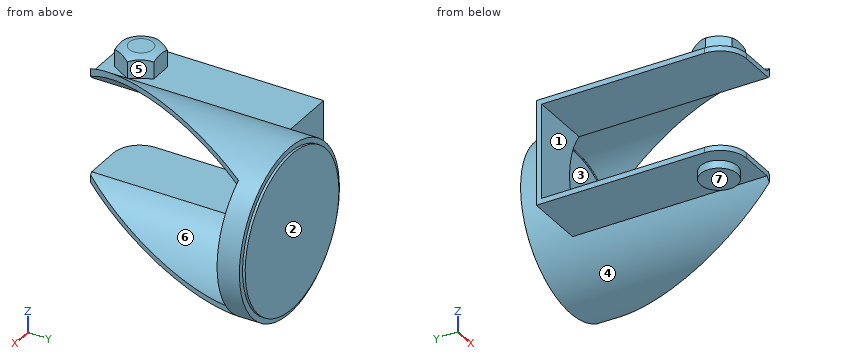
from build123d import *

# Parameters (mm, degrees)
SKETCH2_W               = 36
SKETCH2_H               = 106
CUT_EXTRUDE1_DEPTH      = 95
BOSS_EXTRUDE1_DEPTH     = 47.5
SKETCH4_R               = 29.766666667
CUT_EXTRUDE2_DEPTH      = 144
CUT_EXTRUDE3_DEPTH      = 95
CUT_EXTRUDE3_DEPTH_BACK = 95
SKETCH6_R               = 7
BOSS_EXTRUDE2_DEPTH     = 3
SKETCH8_R               = 9
CUT_EXTRUDE4_DEPTH      = 10


with BuildPart() as part:
    # Sketch1 → Revolve1 (revolve)
    with BuildSketch(Plane(origin=(0, 0, 0), x_dir=(0, 0, -1), z_dir=(1, 0, 0))):
        Polygon((0, -17.975), (-29.666666667, -17.975), (-29.666666667, -109.475), (-31.666666667, -109.475), (-31.666666667, -16.475), (-29.666666667, -16.475), (-29.666666667, -15.475), (0, -15.475), align=None)
    revolve(axis=Axis((0, -15.475, 0), (0, -1, 0)))

    # Sketch2 → Cut-Extrude1 (cut)
    with BuildSketch(Plane(origin=(0, 0, 0), x_dir=(0, 0, -1), z_dir=(1, 0, 0))):
        with Locations((0, -87)):
            Rectangle(SKETCH2_W, SKETCH2_H)
    extrude(amount=-CUT_EXTRUDE1_DEPTH, mode=Mode.SUBTRACT)

    # Sketch3 → Boss-Extrude1 (add)
    with BuildSketch(Plane(origin=(0, 0, 0), x_dir=(0, 0, -1), z_dir=(1, 0, 0))):
        Polygon((-20, -32), (-20, -106), (-18, -106), (-18, -34), (18, -34), (18, -106), (20, -106), (20, -32), align=None)
    extrude(amount=-BOSS_EXTRUDE1_DEPTH)

    # Sketch4 → Cut-Extrude2 (cut)
    with BuildSketch(Plane(origin=(0, -18.475, 0), x_dir=(1, 0, 0), z_dir=(0, 1, 0))):
        with Locations(Location((0, 0, 0), (0, 0, 270))):
            Circle(SKETCH4_R)
    extrude(amount=-CUT_EXTRUDE2_DEPTH, mode=Mode.SUBTRACT)

    # Sketch5 → Cut-Extrude3 (cut, two sides: drawn at the far end of the back side and taken through both)
    with BuildSketch(Plane.XY.offset(-CUT_EXTRUDE3_DEPTH_BACK)):
        with BuildLine():
            Line((-81.666666667, -159.475), (31.666666667, -159.475))
            Line((31.666666667, -159.475), (31.666666667, -24.975))
            Line((31.666666667, -24.975), (18.095238095, -24.975))
            Line((18.095238095, -24.975), (-23.03030303, -106))
            Line((-23.03030303, -106), (-37.5, -106))
            ThreePointArc((-37.5, -106), (-44.571067812, -103.071067812), (-47.5, -96))
            Line((-47.5, -96), (-47.5, -61.653061224))
            Line((-47.5, -61.653061224), (-81.666666667, -106))
            Line((-81.666666667, -106), (-81.666666667, -159.475))
        make_face()
    extrude(amount=CUT_EXTRUDE3_DEPTH + CUT_EXTRUDE3_DEPTH_BACK, mode=Mode.SUBTRACT)

    # Sketch6 → Boss-Extrude2 (add)
    with BuildSketch(Plane.XY.offset(-20)):
        with Locations((-35, -94)):
            Circle(SKETCH6_R)
    extrude(amount=-BOSS_EXTRUDE2_DEPTH)

    # Sketch7 → Revolve2 (revolve)
    with BuildSketch(Plane(origin=(-35, 0, 0), x_dir=(0, 0, -1), z_dir=(1, 0, 0)), mode=Mode.PRIVATE) as revolve2_sk:
        with BuildLine():
            Line((-28, -94), (-28, -89.5))
            ThreePointArc((-28, -89.5), (-27.442646012, -87.053268439), (-26, -85))
            Line((-26, -85), (-20, -85))
            Line((-20, -85), (-20, -94))
            Line((-20, -94), (-28, -94))
        make_face()
    revolve(revolve2_sk.sketch.rotate(Axis((-35, -94, 20), (0, 0, 1)), 90), axis=Axis((-35, -94, 20), (0, 0, 1)))

    # Sketch8 → Cut-Extrude4 (cut)
    with BuildSketch(Plane.XY.offset(20)):
        with Locations((-35, -94)):
            Circle(SKETCH8_R)
        Polygon((-43.660254038, -94), (-39.330127019, -101.5), (-30.669872981, -101.5), (-26.339745962, -94), (-30.669872981, -86.5), (-39.330127019, -86.5), align=None, mode=Mode.SUBTRACT)
    extrude(amount=CUT_EXTRUDE4_DEPTH, mode=Mode.SUBTRACT)


solid = part.part
Build history of the part. All positions in model axes, mm. Face numbers are marked on the shaded views. A direction names the side the tool comes from. Coordinates: 2 decimals unless noted, no trailing zeros. Order: outer loops, then holes, each group sorted by start corner. A loop starts at its lowest first (then second) coordinate and runs counter-clockwise, first axis right, second up. Notation, with made-up numbers: (33.25, 16.25) - (90.25, 16.25) arc R34 cw to (90.25, 54.25) - close; hole circle Ø7 at (-13.75, -7.75). An arc over 180 degrees is marked (long way). Write each question's results on one line, items separated by ' | '. Start each with the question number.
Item 1: Band-saw the part on A-A on z = 0. Write the cut outline in (x, y) (3 decimals).
Item 2: Mould opens along X. For the marked faces 6 and 7 say: released by +X, released by -X, zero draft, split by the parting line, or undercut.
Item 3: Flat gauge pins, fed straight in: pin 1 (3 mm diameter, centred on x = -15.5, y = -35.5, fed in from +Z); pin 2 (25 mm diameter, centred on x = -39, y = -67, fed in from -Z); pin 3 (12 mm diameter, centred on x = -38, z = -7.5, fed in from -Y). Where does each tip first touch, or does it go through?
Item 4: Wall check: probe 1 along Z at (x, y) = (0, -46); probe 2 along Z at (x, y) = (-25.5, -98); probe 3 along X at (y, z) = (-18.3, 0). Give the ranges that are in metal, low to high. Write a range as [from, to].
Item 5: Band-saw the part on C-C on x = 0. Write the cut outline in (y, z) (3 decimals), and give its area (3 significant figures).
Item 6: Tool access for the marked faces 1, 2, 3, 4 and 5: list every direction of +Z, -Z, +X, -X, +Y, -Y with a clear straight run to the whole face (end or side of a thin tool).
Item 7: Band-saw the part on D-D on y = -62. Write the cut outline in (x, z), and give its area (3 significant figures).
Item 8: Band-saw the part on B-B on y = -45. Write the cut outline in (x, z), and give its area (3 significant figures).
Numbers:
1) outline: (-47.5, -34) - (-29.767, -34) - (-29.767, -18.475) - (-29.667, -18.475) - (-29.667, -17.975) - (29.667, -17.975) - (29.667, -18.475) - (29.767, -18.475) - (29.767, -24.975) - (31.667, -24.975) - (31.667, -16.475) - (29.667, -16.475) - (29.667, -15.475) - (-29.667, -15.475) - (-29.667, -16.475) - (-31.667, -16.475) - (-31.667, -32) - (-47.5, -32) - close
2) face 6: undercut | face 7: zero draft
3) pin 1: z = 28.4 | pin 2: z = -20 | pin 3: y = -34
4) probe 1: [-31.67, -29.77], [29.77, 31.67] | probe 2: [-20, -18], [18, 20] | probe 3: [-31.67, -29.67], [29.67, 31.67]
5) outline: (-60.626, -31.667) - (-16.475, -31.667) - (-16.475, -29.667) - (-15.475, -29.667) - (-15.475, 29.667) - (-16.475, 29.667) - (-16.475, 31.667) - (-60.626, 31.667) - (-60.626, 29.767) - (-18.475, 29.767) - (-18.475, 29.667) - (-17.975, 29.667) - (-17.975, -29.667) - (-18.475, -29.667) - (-18.475, -29.767) - (-60.626, -29.767) - close | area: 317 mm^2
6) face 1: +X, -X, -Y | face 2: +Z, -Z, +X, -X, +Y | face 3: -Y | face 4: +Y | face 5: +Z, +Y
7) outline: (-47.5, -20) - (-24.55, -20) arc R31.67 ccw to (-0.7, -31.66) - (-0.7, -29.76) arc R29.77 cw to (-23.71, -18) - (-47.5, -18) - close; (-47.5, 18) - (-23.71, 18) arc R29.77 cw to (-0.7, 29.76) - (-0.7, 31.66) arc R31.67 ccw to (-24.55, 20) - (-47.5, 20) - close | area: 196 mm^2
8) outline: (-47.5, -20) - (-24.55, -20) arc R31.67 ccw to (7.93, -30.66) - (7.93, -28.69) arc R29.77 cw to (-23.71, -18) - (-47.5, -18) - close; (-47.5, 18) - (-23.71, 18) arc R29.77 cw to (7.93, 28.69) - (7.93, 30.66) arc R31.67 ccw to (-24.55, 20) - (-47.5, 20) - close | area: 229 mm^2
